from build123d import *

# Parameters (mm, degrees)
BOSS_EXTRUDE1_DEPTH        = 2.3
SKETCH2_W                  = 42
SKETCH2_H                  = 2.3
BOSS_EXTRUDE2_DEPTH        = 7.7
F_10_0_10_DIAMETER_HOLE1_D = 10
F_5_5_5_5_DIAMETER_HOLE1_D = 5.5
CHAMFER1_SIZE              = 13.335010311


with BuildPart() as part:
    # Sketch1 → Boss-Extrude1 (new body)
    with BuildSketch(Plane(origin=(-2.3, 0, 0), x_dir=(0, -1, 0), z_dir=(-1, 0, 0))):
        Polygon((11.7, 21), (-22.35, 0), (11.7, -21), (14, -21), (14, 21), align=None)
    extrude(amount=-BOSS_EXTRUDE1_DEPTH)

    # Sketch2 → Boss-Extrude2 (add)
    with BuildSketch(Plane.ZY.offset(2.3)):
        with Locations((0, -12.85)):
            Rectangle(SKETCH2_W, SKETCH2_H)
    extrude(amount=BOSS_EXTRUDE2_DEPTH)

    # Ø10.0 (10) Diameter Hole1 (through all)
    with Locations(Plane.ZY.offset(2.3)):
        with Locations((0, 0)):
            Hole(F_10_0_10_DIAMETER_HOLE1_D / 2)

    # Ø5.5 (5.5) Diameter Hole1 (through all)
    with Locations(Plane(origin=(0, -11.7, 0), x_dir=(1, 0, 0), z_dir=(0, 1, 0))):
        with Locations((-6, -16.5), (-6, 16.5)):
            Hole(F_5_5_5_5_DIAMETER_HOLE1_D / 2)

    # Chamfer1
    chamfer1_edges = [part.edges().sort_by_distance(p)[0] for p in [
        (-1.15, 22.35, 0),
    ]]
    chamfer(chamfer1_edges, length=CHAMFER1_SIZE)


solid = part.part
Input: part model. Units: mm. Frame: model coordinates. A direction names the side the tool comes from. Give positions to 0.01 mm unless a question says otherwise; leave off trailing zeros. Order: outer loops, then holes, each group sorted by start corner. A loop starts at its lowest first (then second) coordinate and runs counter-clockwise, first axis right, second up. Notation, with made-up numbers: M 50,-23 L 74,-23 A29 cw 74,2 Z; hole C 11,80.5 d9. An arc over 180 degrees is marked long. Answer as a JSON object with one key per item and string values.
1. First-contact query: P1, Ø1, axis at y = -5, z = 4.5, coming from the -X side; P2, Ø2.5, axis at x = -8, z = 0, coming from the +Y side; P3, Ø9, axis at y = 0, z = 0, coming from the +X side. Flat tips, straight axial feed; report the tip coordinate or a pass-through.
Result sheet:
{"P1": "x = -2.3", "P2": "y = -11.7", "P3": "through"}
2. Cut plane A-A, the plane z = 0. Output: boundary loops of the cut face in (x, y), and give its area (3 significant figures).
Result sheet:
{"outline": "M -10,-14 L 0,-14 L 0,-5 L -2.3,-5 L -2.3,-11.7 L -10,-11.7 Z; M -2.3,5 L 0,5 L 0,11 L -2.3,11 Z", "area": "52.2 mm²"}
3. Pull-direction query (Z, two-part tool) for faces 3 (the flat face through (-6, -11.7, 0)), 4 (the flat face through (-1.17, -0.51, 14.1)), 5 (the cylindrical face through (-5.642, -12.866, -19.227)); classes: +Z half, -Z half, draft (parallel to the pull), parting line (faces both ways), or undercut.
Result sheet:
{"face 3": "draft", "face 4": "+Z half", "face 5": "undercut"}
4. Ray query, line 1 (Z direction, x = -6, y = -12.55); line 2 (X direction, y = -13.25, z = -16.5); line 3 (Y direction, x = -8, z = 19). Return the intervals inside material, ascending. Write a range as [from, to].
Result sheet:
{"line 1": "[-21, -19.25], [-13.75, 13.75], [19.25, 21]", "line 2": "[-10, -8.75], [-3.25, 0]", "line 3": "[-14, -11.7]"}
5. Cut plane D-D, the plane x = -1.5. Output: boundary loops of the cut face in (y, z).
Result sheet:
{"outline": "M -14,-21 L -11.7,-21 L 11,-7 L 11,7 L -11.7,21 L -14,21 Z; hole C 0,0 d10"}
6. Reachability of faces 1 (the flat face through (-2.3, -5.2, 0.3)), 2 (the flat face through (-1, 11, 0)) from +Z, -Z, +X, -X, +Y, -Y: full face, straight path, thin tool, end or side. Return the list, or none.
Result sheet:
{"face 1": "+Z, -Z, -X, +Y", "face 2": "+Z, -Z, +X, -X, +Y"}
7. Cut plane B-B, the plane x = -6. Output: boundary loops of the cut face in (y, z).
Result sheet:
{"outline": "M -14,-21 L -11.7,-21 L -11.7,-19.25 L -14,-19.25 Z; M -14,-13.75 L -11.7,-13.75 L -11.7,13.75 L -14,13.75 Z; M -14,19.25 L -11.7,19.25 L -11.7,21 L -14,21 Z"}
8. Cut plane C-C, the plane y = 2.75. Output: boundary loops of the cut face in (x, z), and give its area (3 significant figures).
Result sheet:
{"outline": "M -2.3,-12.09 L 0,-12.09 L 0,-4.18 L -2.3,-4.18 Z; M -2.3,4.18 L 0,4.18 L 0,12.09 L -2.3,12.09 Z", "area": "36.4 mm²"}
